Geometry: final body of the model. Coordinates: model frame, mm. Give positions to 0.01 mm unless a question says otherwise; leave off trailing zeros. Loops run counter-clockwise (first coordinate to the right, second up) from the corner with the lowest first, then second, coordinate; pieces in that order, holes last. Notation, with made-up numbers: (-34.75, 49) - (8.25, 49) arc R28 ccw to (8.25, 67) - close; hole circle Ø11 at (12, 80.5). An arc over 180 degrees is marked (long way). Use one line per item in the form item = value.
```python
from build123d import *

# Parameters (mm, degrees)
EXTRUDE_1_DEPTH             = 20
HOLE_WIZARD_M3_1_AT_2_COUNT = 2
HOLE_WIZARD_M3_1_AT_2_PITCH = 10
FILLET_1_R                  = 1


with BuildPart() as part:
    # 草图1 → 凸台-拉伸1 (new body)
    with BuildSketch(Plane(origin=(0, 0, 0), x_dir=(1, 0, 0), z_dir=(0, 1, 0))):
        Polygon((0, 0), (15, 0), (18.882285677, 14.488887394), align=None)
    extrude(amount=EXTRUDE_1_DEPTH)

    # 草图4 → M3 螺纹孔1 (revolve, cut)
    with BuildSketch(Plane(origin=(17.070552361, 15, -7.72740661), x_dir=(0.25881904510251796, 0, -0.9659258262890691), z_dir=(0, 1, 0))):
        Polygon((0, 0), (0, 7.5), (1.25, 6.748924226), (1.25, 0), align=None)
    hole_wizard_m3_1 = revolve(axis=Axis((23.204181358, 15, -6.083905674), (-0.9659258262890691, 0, -0.2588190451025179)), mode=Mode.SUBTRACT)

    # M3 螺纹孔1 at 2: M3 螺纹孔1 ×2
    with Locations(*[(0, -i * HOLE_WIZARD_M3_1_AT_2_PITCH, 0) for i in range(1, HOLE_WIZARD_M3_1_AT_2_COUNT)]):
        add(hole_wizard_m3_1, mode=Mode.SUBTRACT)

    # 镜向1: M3 螺纹孔1 across plane
    add(hole_wizard_m3_1.mirror(Plane(origin=(9.441142838, 0, -7.244443697), x_dir=(0.6087614290087218, 0, 0.7933533402912344), z_dir=(0.7933533402912343, 0, -0.6087614290087218))), mode=Mode.SUBTRACT)

    # 镜向1 copy 1 sketch → 镜向1 copy 1 (revolve, cut)
    with BuildSketch(Plane(origin=(7, 5, 0), x_dir=(-1, 0, 0), z_dir=(0, 1, 0))):
        Polygon((0, 0), (0, -7.5), (1.25, -6.748924226), (1.25, 0), align=None)
    revolve(axis=Axis((7, 5, 6.35), (0, 0, 1)), mode=Mode.SUBTRACT)

    # 圆角1
    fillet_1_edges = [part.edges().sort_by_distance(p)[0] for p in [
        (18.882285677, 10, -14.488887394),
        (15, 10, 0),
        (0, 10, 0),
    ]]
    fillet(fillet_1_edges, radius=FILLET_1_R)


solid = part.part
```
(1) Pin query (flat end, axial travel): P1, Ø1.5, axis at y = 3.5, z = -4, coming from the +X side; P2, Ø1, axis at x = 15, y = 9, coming from the -Z side; P3, Ø1.5, axis at x = 7, y = 5, coming from the -Z side. Return the tip coordinate at first contact, or that it passes through.
Solution:
P1 = 16.27
P2 = -11.89
P3 = through
(2) Cut plane C-C (y = 15.75). Return the cut outline in (x, z).
Solution:
outline = (2.34, -1.79) - (6, -4.6) - (6, 0) - (2.95, 0) arc R1 ccw to start; (8, -6.14) - (10.88, -8.35) - (16.81, -6.76) - (15.2, -0.74) arc R1 ccw to (14.23, 0) - (8, 0) - close; (12.88, -9.88) - (16.55, -12.7) arc R1 ccw to (18.12, -11.64) - (17.33, -8.69) - close
(3) Pull-direction query (Y, two-part tool) for faces 1 (the face through (12, 0, -5)), 2 (the face through (14.83, 10.14, -0.2)), 3 (the face through (14.379, 14.945, -7.156)); classes: released by +Y, released by -Y, zero draft, split by the parting line, or undercut.
Solution:
face_1 = released by -Y
face_2 = zero draft
face_3 = undercut
(4) Cut plane B-B (y = 7.75). Return the cut outline in (x, z), plus the area to 3 significant figures.
Solution:
outline = (2.34, -1.79) - (16.55, -12.7) arc R1 ccw to (18.12, -11.64) - (15.2, -0.74) arc R1 ccw to (14.23, 0) - (2.95, 0) arc R1 ccw to start
area = 105 mm2
(5) Cut plane D-D (z = -8.25). Give the number of separate pieces and of enclosed holes in the cut face, plus the area to 3 significant figures.
Solution:
separate_pieces = 3
enclosed_holes = 0
area = 101 mm2
(6) Material intervals for L1, parallel to Y at x = 7, z = -4.5; L2, parallel to Y at x = 13.5, z = -9.5; L3, parallel to X at y = 15, z = -3, sorted ascending. Write a range as from..to.
Solution:
L1 = 0..3.75, 6.25..13.75, 16.25..20
L2 = 0..4.03, 5.97..14.03, 15.97..20
L3 = 3.91..5.75, 8.25..15.8
(7) Cut plane A-A (x = 7). Return the cut outline in (y, z), plus the area to 3 significant figures.
Solution:
outline = (0, -5.37) - (3.75, -5.37) - (3.75, 0) - (0, 0) - close; (6.25, -5.37) - (13.75, -5.37) - (13.75, 0) - (6.25, 0) - close; (16.25, -5.37) - (20, -5.37) - (20, 0) - (16.25, 0) - close
area = 80.6 mm2
